from build123d import *

# Parameters (mm, degrees)
SKETCH1_R             = 21.5
BOSS_EXTRUDE1_DEPTH   = 37
SKETCH2_R             = 24
BOSS_EXTRUDE2_DEPTH   = 15
SKETCH3_R             = 22
BOSS_EXTRUDE3_DEPTH   = 21
SKETCH4_R             = 9
BOSS_EXTRUDE4_DEPTH   = 16
SKETCH5_R             = 7
BOSS_EXTRUDE5_DEPTH   = 17
CUT_EXTRUDE1_START    = 30
CUT_EXTRUDE1_DEPTH    = 25
BOSS_EXTRUDE6_START   = 38
SKETCH7_R             = 21.5
BOSS_EXTRUDE6_DEPTH   = 38
SKETCH9_R             = 31
BOSS_EXTRUDE7_DEPTH   = 5
M8_TAPPED_HOLE1_D     = 6.8
M8_TAPPED_HOLE1_DEPTH = 35
M8_TAPPED_HOLE1_TIP   = 2.042926105


with BuildPart() as part:
    # Sketch1 → Boss-Extrude1 (new body)
    with BuildSketch(Plane.XY.offset(38)):
        Circle(SKETCH1_R)
    extrude(amount=BOSS_EXTRUDE1_DEPTH)

    # Sketch2 → Boss-Extrude2 (add)
    with BuildSketch(Plane.XY.offset(75)):
        Circle(SKETCH2_R)
    extrude(amount=BOSS_EXTRUDE2_DEPTH)

    # Sketch3 → Boss-Extrude3 (add)
    with BuildSketch(Plane.XY.offset(90)):
        Circle(SKETCH3_R)
    extrude(amount=BOSS_EXTRUDE3_DEPTH)

    # Sketch4 → Boss-Extrude4 (add)
    with BuildSketch(Plane.XY.offset(111)):
        Circle(SKETCH4_R)
    extrude(amount=BOSS_EXTRUDE4_DEPTH)

    # Sketch5 → Boss-Extrude5 (add)
    with BuildSketch(Plane.XY.offset(127)):
        Circle(SKETCH5_R)
    extrude(amount=BOSS_EXTRUDE5_DEPTH)

    # Sketch6 → Cut-Extrude1 (cut)
    with BuildSketch(Plane(origin=(0, 0, 0), x_dir=(1, 0, 0), z_dir=(0, 1, 0)).offset(CUT_EXTRUDE1_START)):
        with BuildLine():
            Line((1.85, -130.63993085), (1.85, -140.5))
            ThreePointArc((1.85, -140.5), (0, -142.35), (-1.85, -140.5))
            Line((-1.85, -140.5), (-1.85, -130.63993085))
            ThreePointArc((-1.85, -130.63993085), (0, -128.78993085), (1.85, -130.63993085))
        make_face()
    extrude(amount=-CUT_EXTRUDE1_DEPTH, mode=Mode.SUBTRACT)

    # Sketch7 → Boss-Extrude6 (add)
    with BuildSketch(Plane(origin=(0, 0, 38), x_dir=(-1, 0, 0), z_dir=(0, 0, -1)).offset(BOSS_EXTRUDE6_START)):
        Circle(SKETCH7_R)
    extrude(amount=-BOSS_EXTRUDE6_DEPTH)

    # Sketch9 → Boss-Extrude7 (add)
    with BuildSketch(Plane.XY.offset(38)):
        Circle(SKETCH9_R)
    extrude(amount=BOSS_EXTRUDE7_DEPTH)

    # M8 Tapped Hole1
    with Locations(Plane(origin=(0, 0, 0), x_dir=(-1, 0, 0), z_dir=(0, 0, -1))):
        with Locations((0, 0)):
            Hole(M8_TAPPED_HOLE1_D / 2, depth=M8_TAPPED_HOLE1_DEPTH)
            with Locations((0, 0, -(M8_TAPPED_HOLE1_DEPTH + M8_TAPPED_HOLE1_TIP / 2))):  # 118° drill point
                Cone(0, M8_TAPPED_HOLE1_D / 2, M8_TAPPED_HOLE1_TIP, mode=Mode.SUBTRACT)


solid = part.part
Input: part model. Units: mm. Frame: model coordinates. A direction names the side the tool comes from. Round coordinates to 2 decimals unless told otherwise and drop trailing zeros. Loops run counter-clockwise (first coordinate to the right, second up) from the corner with the lowest first, then second, coordinate; pieces in that order, holes last. Notation, with made-up numbers: M 44.25,-39.5 L 52.25,-39.5 A31 cw 52.25,-10.5 Z; hole C 23,27 d2. An arc over 180 degrees is marked long. Answer as CSV lines item,"result". Start each with the question number.
(1) Line query: line 1 (Y direction, x = 0, z = 16.5); line 2 (Z direction, x = 4.5, y = 23). Output: solid intervals per line, ascending. Write a range as [from, to].
(2) First-contact query: pin 1 (12 mm diameter, centred on y = 4.5, z = 103.5, fed in from -X); pin 2 (12 mm diameter, centred on x = -15.5, z = 28, fed in from +Y); pin 3 (4 mm diameter, centred on y = 3, z = 40, fed in from +X). Flat tips, straight axial feed; report the tip coordinate or a pass-through.
(3) Section D-D, the plane x = 5.5. Output: boundary loops of the cut face in (y, z).
(4) Section A-A, the plane y = 20. Output: boundary loops of the cut face in (x, z), plus the area to 3 significant figures.
(5) Section B-B, the plane z = 134. Output: boundary loops of the cut face in (x, y), plus the area to 3 significant figures.
(6) Draft query along X for faces 1 (the conical face through (0.128, -0.576, 36.688)), 2 (the flat face through (7, -21.2, 90)), 3 (the cylindrical face through (-2.799, 21.317, 58.776)). Return one class per face: released by +X, released by -X, zero draft, split by the parting line, or undercut.
(7) Reachability of faces 4 (the cylindrical face through (-23.977, 1.055, 82.395)), 5 (the cylindrical face through (-0.74, -3.32, 17.75)), 6 (the flat face through (-20, 9, 75)) from +Z, -Z, +X, -X, +Y, -Y: full face, straight path, thin tool, end or side. Return the list, or none.
Values found:
1,line 1,"y = [-21.5, -3.4], [3.4, 21.5]"
1,line 2,"z = [38, 43], [75, 90]"
2,pin 1,"stops at x = -22"
2,pin 2,"stops at y = 19.29"
2,pin 3,"stops at x = 30.98"
3,outline,"M -30.51,38 L -20.78,38 L -20.78,0 L 20.78,0 L 20.78,38 L 30.51,38 L 30.51,43 L 20.78,43 L 20.78,75 L 23.36,75 L 23.36,90 L 21.3,90 L 21.3,111 L 7.12,111 L 7.12,127 L 4.33,127 L 4.33,144 L -4.33,144 L -4.33,127 L -7.12,127 L -7.12,111 L -21.3,111 L -21.3,90 L -23.36,90 L -23.36,75 L -20.78,75 L -20.78,43 L -30.51,43 Z"
4,outline,"M -23.69,38 L -7.89,38 L -7.89,0 L 7.89,0 L 7.89,38 L 23.69,38 L 23.69,43 L 7.89,43 L 7.89,75 L 13.27,75 L 13.27,90 L 9.17,90 L 9.17,111 L -9.17,111 L -9.17,90 L -13.27,90 L -13.27,75 L -7.89,75 L -7.89,43 L -23.69,43 Z"
4,area,"2,120 mm²"
5,outline,"M -1.85,5 L -1.85,6.75 A7 ccw long 1.85,6.75 L 1.85,5 Z"
5,area,"147 mm²"
6,face 1,"undercut"
6,face 2,"zero draft"
6,face 3,"split by the parting line"
7,face 4,"+Z"
7,face 5,"-Z"
7,face 6,"none"
